Part model, mm, in its own coordinate system. Face numbers are marked on the shaded views. Coordinates: 2 decimals unless noted, no trailing zeros. Order: outer loops, then holes, each group sorted by start corner. A loop starts at its lowest first (then second) coordinate and runs counter-clockwise, first axis right, second up.
from build123d import *

# Parameters (mm, degrees)
SWEEP_THIN_PART_1_PROFILE_R   = 10
SWEEP_THIN_PART_1_PROFILE_R_2 = 7.5
SWEEP_THIN_PART_2_PROFILE_R   = 10
SWEEP_THIN_PART_2_PROFILE_R_2 = 7.5
SKETCH15_R                    = 7.5
CUT_EXTRUDE1_DEPTH            = 62.67049551
SKETCH18_R                    = 7.5
CUT_EXTRUDE2_DEPTH            = 30


with BuildPart() as part:
    # Sweep-thin part 1: sweep along a path in Sketch1
    with BuildLine(Plane.XY) as sweep_thin_part_1_path:
        Line((-26.75, 0), (26.75, 0))
    # Sweep-thin part 1 profile (on start of the path) → Sweep-thin part 1 (sweep)
    with BuildSketch(Plane.YZ.offset(-26.75)):
        Circle(SWEEP_THIN_PART_1_PROFILE_R)
        Circle(SWEEP_THIN_PART_1_PROFILE_R_2, mode=Mode.SUBTRACT)
    sweep(path=sweep_thin_part_1_path.line)

    # Sweep-thin part 2: sweep along a path in Sketch8
    with BuildLine(Plane.XY) as sweep_thin_part_2_path:
        Line((0, 0), (0, -29))
    # Sweep-thin part 2 profile (on start of the path) → Sweep-thin part 2 (sweep)
    with BuildSketch(Plane(origin=(0, 0, 0), x_dir=(-1, 0, 0), z_dir=(0, -1, 0))):
        Circle(SWEEP_THIN_PART_2_PROFILE_R)
        Circle(SWEEP_THIN_PART_2_PROFILE_R_2, mode=Mode.SUBTRACT)
    sweep(path=sweep_thin_part_2_path.line)

    # Sketch15 → Cut-Extrude1 (cut, through all)
    with BuildSketch(Plane.ZY.offset(26.75)):
        with Locations(Location((0, 0, 0), (0, 0, 90))):
            Circle(SKETCH15_R)
    extrude(amount=-CUT_EXTRUDE1_DEPTH, mode=Mode.SUBTRACT)

    # Sketch18 → Cut-Extrude2 (cut)
    with BuildSketch(Plane.XZ.offset(29)):
        Circle(SKETCH18_R)
    extrude(amount=-CUT_EXTRUDE2_DEPTH, mode=Mode.SUBTRACT)


solid = part.part
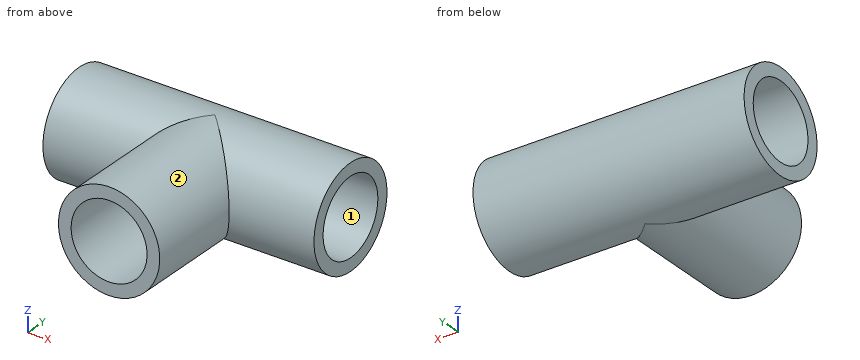
Q1. Wall check: line 1 along X through (y, z) = (-20.5, 0). Give the ranges that are in metal, low to high.
Results list:
line 1: x = -10 to -7.5, 7.5 to 10
Q2. Cut at D-D on x = -18. Write the cut outline in (y, z).
Results list:
outline: circle Ø20 at (0, 0); hole circle Ø15 at (0, 0)
Q3. Pin check, flat tips, straight feed: pin 1 Ø4 at (x, z) = (-3.5, 1) entering from -Y; pin 2 Ø1.5 at (x, y) = (3.5, -6.5) entering from -Z; pin 3 Ø9 at (x, z) = (0, 0) entering from -Y; pin 4 Ø4 at (x, y) = (12.5, -21.5) entering from +Z. Stop position of each tip, or through.
Results list:
pin 1: stops at y = 6.87
pin 2: stops at z = -9.61
pin 3: stops at y = 6
pin 4: passes through
Q4. Mould opens along Z. For the marked faces 1 and 2 say: pulls with the +Z half, pulls with the -Z half, needs draft (parallel to the pull), parting line crosses it, or undercut.
Results list:
face 1: undercut
face 2: parting line crosses it
Q5. Cut at A-A on z = 0. Write the cut outline in (x, y), and give its area (3 significant figures).
Results list:
outline: (-26.75, -10) - (-10, -10) - (-10, -29) - (-7.5, -29) - (-7.5, -7.5) - (-26.75, -7.5) - close; (-26.75, 7.5) - (26.75, 7.5) - (26.75, 10) - (-26.75, 10) - close; (7.5, -29) - (10, -29) - (10, -10) - (26.75, -10) - (26.75, -7.5) - (7.5, -7.5) - close
area: 325 mm2
Q6. Cut at B-B on y = 4.5. Write the cut outline in (x, z).
Results list:
outline: (-26.75, -8.93) - (26.75, -8.93) - (26.75, -6) - (-26.75, -6) - close; (-26.75, 6) - (26.75, 6) - (26.75, 8.93) - (-26.75, 8.93) - close
Q7. Cut at C-C on x = 3. Write the cut outline in (y, z).
Results list:
outline: (-29, -9.54) - (-3, -9.54) arc R10 ccw (long way) to (-3, 9.54) - (-29, 9.54) - (-29, 6.87) - (-3, 6.87) arc R7.5 cw (long way) to (-3, -6.87) - (-29, -6.87) - close
